from build123d import *

# Parameters (mm, degrees)
SKETCH1_W             = 100
SKETCH1_H             = 50
BOSS_EXTRUDE1_DEPTH   = 10
FILLET1_R             = 10
M6_TAPPED_HOLE1_D     = 5
M6_TAPPED_HOLE1_DEPTH = 13.497848452
M6_TAPPED_HOLE1_TIP   = 1.502151548
SKETCH2_W             = 40
SKETCH2_H             = 50
CUT_EXTRUDE1_DEPTH    = 5


with BuildPart() as part:
    # Sketch1 → Boss-Extrude1 (new body)
    with BuildSketch(Plane(origin=(0, 0, 0), x_dir=(1, 0, 0), z_dir=(0, 1, 0))):
        Rectangle(SKETCH1_W, SKETCH1_H)
    extrude(amount=BOSS_EXTRUDE1_DEPTH)

    # Fillet1
    fillet1_edges = [part.edges().sort_by_distance(p)[0] for p in [
        (50, 5, 25),
        (-50, 5, 25),
        (-50, 5, -25),
        (50, 5, -25),
    ]]
    fillet(fillet1_edges, radius=FILLET1_R)

    # M6 Tapped Hole1
    with Locations(Plane(origin=(-40, 10, 15), x_dir=(0, 0, 1), z_dir=(0, 1, 0))):
        with Locations((0, 0), (-30, 0), (-30, 80), (0, 80)):
            Hole(M6_TAPPED_HOLE1_D / 2, depth=M6_TAPPED_HOLE1_DEPTH)
            with Locations((0, 0, -(M6_TAPPED_HOLE1_DEPTH + M6_TAPPED_HOLE1_TIP / 2))):  # 118° drill point
                Cone(0, M6_TAPPED_HOLE1_D / 2, M6_TAPPED_HOLE1_TIP, mode=Mode.SUBTRACT)

    # Sketch2 → Cut-Extrude1 (cut)
    with BuildSketch(Plane(origin=(0, 10, 0), x_dir=(1, 0, 0), z_dir=(0, 1, 0))):
        Rectangle(SKETCH2_W, SKETCH2_H)
    extrude(amount=-CUT_EXTRUDE1_DEPTH, mode=Mode.SUBTRACT)


solid = part.part
Could you check a few things on this model? Use its own coordinates, in mm. A direction names the side the tool comes from. Give positions to 0.01 mm unless a question says otherwise; leave off trailing zeros. Order: outer loops, then holes, each group sorted by start corner. A loop starts at its lowest first (then second) coordinate and runs counter-clockwise, first axis right, second up.
1. Suppose I cut it at B-B (y = 1). Write out the boundary of the cut face in (x, z).
Answers below:
outline: (-50, -15) arc R10 ccw to (-40, -25) - (40, -25) arc R10 ccw to (50, -15) - (50, 15) arc R10 ccw to (40, 25) - (-40, 25) arc R10 ccw to (-50, 15) - close; hole circle Ø5 at (-40, -15); hole circle Ø5 at (-40, 15); hole circle Ø5 at (40, -15); hole circle Ø5 at (40, 15)
2. Thinking about a two-plate mould opening in X: for faces 1 (the flat face through (-1, 0, 0)), 2 (the cylindrical face through (47.15, 5.07, -21.99)), 3 (the cylindrical face through (-39.9, 4.9, -12.5)), which applies, +X half, -X half, draft (parallel to the pull), parting line (faces both ways), or undercut?
Answers below:
face 1: draft
face 2: +X half
face 3: undercut
3. Suppose I cut it at C-C (z = -8). Write out the boundary of the cut face in (x, y).
Answers below:
outline: (-50, 0) - (50, 0) - (50, 10) - (20, 10) - (20, 5) - (-20, 5) - (-20, 10) - (-50, 10) - close
4. Suppose I cut it at D-D (z = 14). Write out the boundary of the cut face in (x, y).
Answers below:
outline: (-50, 0) - (-42.29, 0) - (-42.29, 10) - (-50, 10) - close; (-37.71, 0) - (37.71, 0) - (37.71, 10) - (20, 10) - (20, 5) - (-20, 5) - (-20, 10) - (-37.71, 10) - close; (42.29, 0) - (50, 0) - (50, 10) - (42.29, 10) - close
5. I need wall thicknesses on L1, parallel to X at y = 3.75, z = -15; L2, parallel to X at y = 6.75, z = -2; L3, parallel to X at y = 1, z = 13. Which ranges of each line are inside material? Lowest first, please.
Answers below:
L1: x = -50 to -42.5, -37.5 to 37.5, 42.5 to 50
L2: x = -50 to -20, 20 to 50
L3: x = -50 to -41.5, -38.5 to 38.5, 41.5 to 50
6. For pin 1 (12 mm diameter, centred on x = 1.5, z = -1.5, fed in from +Y), with a flat end and sliding along its axis, tell me the tip position at first contact or that it passes through.
Answers below:
pin 1: stops at y = 5
7. Which directions (+Z, -Z, +X, -X, +Y, -Y) give clear straight access to the entire face, cutting with the end or side of a thin tool? Please do faces 4 (the flat face through (20, 8, 0)), 5 (the flat face through (-1, 4, -25)).
Answers below:
face 4: +Z, -Z, +Y
face 5: -Z, +X, -X, +Y, -Y
8. Suppose I cut it at A-A (y = 8). Write out the boundary of the cut face in (x, z), plus the area to 3 significant figures.
Answers below:
outline: (-50, -15) arc R10 ccw to (-40, -25) - (-20, -25) - (-20, 25) - (-40, 25) arc R10 ccw to (-50, 15) - close; (20, -25) - (40, -25) arc R10 ccw to (50, -15) - (50, 15) arc R10 ccw to (40, 25) - (20, 25) - close; hole circle Ø5 at (-40, -15); hole circle Ø5 at (-40, 15); hole circle Ø5 at (40, -15); hole circle Ø5 at (40, 15)
area: 2,840 mm2
